from build123d import *

# Parameters (mm, degrees)
BASE_PLATE_PROFILE_SKETCH_R               = 4.1
BASE_PLATE_PROFILE_SKETCH_R_2             = 2.1
BASE_PLATE_7_5MM_DEPTH                    = 7.5
CONNECTOR_RECESS_26_4MM_X_2MM_DEPTH       = 2
CONNECTOR_BORE_AND_SCREW_HOLES_REACH      = 47.058
CONNECTOR_BORE_AND_SCREW_HOLES_SKETCH_R   = 8.05
CONNECTOR_BORE_AND_SCREW_HOLES_SKETCH_R_2 = 2.1


with BuildPart() as part:
    # Base Plate Profile Sketch → Base Plate 7.5mm (new body)
    with BuildSketch(Plane(origin=(0, 0, 0), x_dir=(1, 0, 0), z_dir=(0, 1, 0))):
        with BuildLine():
            Line((-34.1, 20), (-34.1, 18.5))
            ThreePointArc((-34.1, 18.5), (-30, 14.4), (-25.9, 18.5))
            Line((-25.9, 18.5), (-25.9, 20))
            Line((-25.9, 20), (25.9, 20))
            Line((25.9, 20), (25.9, 18.5))
            ThreePointArc((25.9, 18.5), (30, 14.4), (34.1, 18.5))
            Line((34.1, 18.5), (34.1, 20))
            Line((34.1, 20), (36, 20))
            ThreePointArc((36, 20), (38.828427125, 18.828427125), (40, 16))
            Line((40, 16), (40, -16))
            ThreePointArc((40, -16), (38.828427125, -18.828427125), (36, -20))
            Line((36, -20), (34.1, -20))
            Line((34.1, -20), (34.1, -18.5))
            ThreePointArc((34.1, -18.5), (30, -14.4), (25.9, -18.5))
            Line((25.9, -18.5), (25.9, -20))
            Line((25.9, -20), (-25.9, -20))
            Line((-25.9, -20), (-25.9, -18.5))
            ThreePointArc((-25.9, -18.5), (-30, -14.4), (-34.1, -18.5))
            Line((-34.1, -18.5), (-34.1, -20))
            Line((-34.1, -20), (-36, -20))
            ThreePointArc((-36, -20), (-38.828427125, -18.828427125), (-40, -16))
            Line((-40, -16), (-40, 16))
            ThreePointArc((-40, 16), (-38.828427125, 18.828427125), (-36, 20))
            Line((-36, 20), (-34.1, 20))
        make_face()
        with Locations(Location((-30, 0, 0), (0, 0, 270))):
            Circle(BASE_PLATE_PROFILE_SKETCH_R, mode=Mode.SUBTRACT)
        with Locations(Location((30, 0, 0), (0, 0, 90))):
            Circle(BASE_PLATE_PROFILE_SKETCH_R, mode=Mode.SUBTRACT)
        with Locations(Location((-20, 0, 0), (0, 0, 270))):
            Circle(BASE_PLATE_PROFILE_SKETCH_R_2, mode=Mode.SUBTRACT)
        with Locations(Location((20, 0, 0), (0, 0, 90))):
            Circle(BASE_PLATE_PROFILE_SKETCH_R_2, mode=Mode.SUBTRACT)
    extrude(amount=BASE_PLATE_7_5MM_DEPTH)

    # Connector Recess Sketch → Connector Recess 26.4mm x 2mm (cut)
    with BuildSketch(Plane(origin=(0, 7.5, 0), x_dir=(1, 0, 0), z_dir=(0, 1, 0))):
        with BuildLine():
            Line((-9.2, -13.2), (9.2, -13.2))
            ThreePointArc((9.2, -13.2), (12.028427125, -12.028427125), (13.2, -9.2))
            Line((13.2, -9.2), (13.2, 9.2))
            ThreePointArc((13.2, 9.2), (12.028427125, 12.028427125), (9.2, 13.2))
            Line((9.2, 13.2), (-9.2, 13.2))
            ThreePointArc((-9.2, 13.2), (-12.028427125, 12.028427125), (-13.2, 9.2))
            Line((-13.2, 9.2), (-13.2, -9.2))
            ThreePointArc((-13.2, -9.2), (-12.028427125, -12.028427125), (-9.2, -13.2))
        make_face()
    extrude(amount=-CONNECTOR_RECESS_26_4MM_X_2MM_DEPTH, mode=Mode.SUBTRACT)

    # Connector Bore and Screw Holes Sketch → Connector Bore and Screw Holes (cut, up to next)
    with BuildSketch(Plane(origin=(0, 5.5, 0), x_dir=(1, 0, 0), z_dir=(0, 1, 0)), mode=Mode.PRIVATE) as connector_bore_and_screw_holes_sk1:
        with Locations(Location((0, 0, 0), (0, 0, 270))):
            Circle(CONNECTOR_BORE_AND_SCREW_HOLES_SKETCH_R)
    connector_bore_and_screw_holes_tool1 = extrude(connector_bore_and_screw_holes_sk1.sketch, amount=-CONNECTOR_BORE_AND_SCREW_HOLES_REACH, mode=Mode.PRIVATE) & part.part
    # Connector Bore and Screw Holes Sketch → Connector Bore and Screw Holes (cut, up to next)
    with BuildSketch(Plane(origin=(0, 5.5, 0), x_dir=(1, 0, 0), z_dir=(0, 1, 0)), mode=Mode.PRIVATE) as connector_bore_and_screw_holes_sk2:
        with Locations(Location((-9.2, 9.2, 0), (0, 0, 270))):
            Circle(CONNECTOR_BORE_AND_SCREW_HOLES_SKETCH_R_2)
    connector_bore_and_screw_holes_tool2 = extrude(connector_bore_and_screw_holes_sk2.sketch, amount=-CONNECTOR_BORE_AND_SCREW_HOLES_REACH, mode=Mode.PRIVATE) & part.part
    # Connector Bore and Screw Holes Sketch → Connector Bore and Screw Holes (cut, up to next)
    with BuildSketch(Plane(origin=(0, 5.5, 0), x_dir=(1, 0, 0), z_dir=(0, 1, 0)), mode=Mode.PRIVATE) as connector_bore_and_screw_holes_sk3:
        with Locations(Location((-9.2, -9.2, 0), (0, 0, 270))):
            Circle(CONNECTOR_BORE_AND_SCREW_HOLES_SKETCH_R_2)
    connector_bore_and_screw_holes_tool3 = extrude(connector_bore_and_screw_holes_sk3.sketch, amount=-CONNECTOR_BORE_AND_SCREW_HOLES_REACH, mode=Mode.PRIVATE) & part.part
    # Connector Bore and Screw Holes Sketch → Connector Bore and Screw Holes (cut, up to next)
    with BuildSketch(Plane(origin=(0, 5.5, 0), x_dir=(1, 0, 0), z_dir=(0, 1, 0)), mode=Mode.PRIVATE) as connector_bore_and_screw_holes_sk4:
        with Locations(Location((9.2, -9.2, 0), (0, 0, 270))):
            Circle(CONNECTOR_BORE_AND_SCREW_HOLES_SKETCH_R_2)
    connector_bore_and_screw_holes_tool4 = extrude(connector_bore_and_screw_holes_sk4.sketch, amount=-CONNECTOR_BORE_AND_SCREW_HOLES_REACH, mode=Mode.PRIVATE) & part.part
    # Connector Bore and Screw Holes Sketch → Connector Bore and Screw Holes (cut, up to next)
    with BuildSketch(Plane(origin=(0, 5.5, 0), x_dir=(1, 0, 0), z_dir=(0, 1, 0)), mode=Mode.PRIVATE) as connector_bore_and_screw_holes_sk5:
        with Locations(Location((9.2, 9.2, 0), (0, 0, 270))):
            Circle(CONNECTOR_BORE_AND_SCREW_HOLES_SKETCH_R_2)
    connector_bore_and_screw_holes_tool5 = extrude(connector_bore_and_screw_holes_sk5.sketch, amount=-CONNECTOR_BORE_AND_SCREW_HOLES_REACH, mode=Mode.PRIVATE) & part.part
    add(connector_bore_and_screw_holes_tool1.solids().sort_by_distance((0, 5.5, 0))[0], mode=Mode.SUBTRACT)
    add(connector_bore_and_screw_holes_tool2.solids().sort_by_distance((-9.2, 5.5, -9.2))[0], mode=Mode.SUBTRACT)
    add(connector_bore_and_screw_holes_tool3.solids().sort_by_distance((-9.2, 5.5, 9.2))[0], mode=Mode.SUBTRACT)
    add(connector_bore_and_screw_holes_tool4.solids().sort_by_distance((9.2, 5.5, 9.2))[0], mode=Mode.SUBTRACT)
    add(connector_bore_and_screw_holes_tool5.solids().sort_by_distance((9.2, 5.5, -9.2))[0], mode=Mode.SUBTRACT)


solid = part.part
CAD build for the part. Positions are in the model's coordinates, mm. A direction names the side the tool comes from. Give positions to 0.01 mm unless a question says otherwise; leave off trailing zeros. Write each loop counter-clockwise with the first axis right and the second up, starting at its lowest first coordinate (ties: lowest second). Pieces come first, ordered by that corner, then holes. Notation, with made-up numbers: (19.25, 2) - (30.25, 2) arc R18 ccw to (30.25, 23) - close; hole circle Ø5 at (14, -13.75). An arc over 180 degrees is marked (long way). Put each result on its own line as item: value.
(1) Saw through at D-D (z = 3). List the corners of the cut face in (x, y).
Working result:
outline: (-40, 0) - (-32.79, 0) - (-32.79, 7.5) - (-40, 7.5) - close; (-27.21, 0) - (-7.47, 0) - (-7.47, 5.5) - (-13.2, 5.5) - (-13.2, 7.5) - (-27.21, 7.5) - close; (7.47, 0) - (27.21, 0) - (27.21, 7.5) - (13.2, 7.5) - (13.2, 5.5) - (7.47, 5.5) - close; (32.79, 0) - (40, 0) - (40, 7.5) - (32.79, 7.5) - close
(2) Tool access for faces 5 (the flat face through (34.1, 4, 19)), 6 (the flat face through (0, 7, -13.2)), 7 (the flat face through (-25.9, 4, -19)): list every direction of +Z, -Z, +X, -X, +Y, -Y with a clear straight run to the whole face (end or side of a thin tool).
Working result:
face 5: +Z, +Y, -Y
face 6: +Y
face 7: -Z, +Y, -Y
(3) Saw through at C-C (x = 30). List the corners of the cut face in (y, z), then the cut area to 4 significant figures.
Working result:
outline: (0, -14.4) - (7.5, -14.4) - (7.5, -4.1) - (0, -4.1) - close; (0, 4.1) - (7.5, 4.1) - (7.5, 14.4) - (0, 14.4) - close
area: 154.5 mm^2
(4) Saw through at A-A (x = -20). List the corners of the cut face in (y, z), then the cut area to 4 significant figures.
Working result:
outline: (0, -20) - (7.5, -20) - (7.5, -2.1) - (0, -2.1) - close; (0, 2.1) - (7.5, 2.1) - (7.5, 20) - (0, 20) - close
area: 268.5 mm^2
(5) Saw through at B-B (y = 2.25). Count the separate pieces of the cut face and the enclosed holes in it, then the cut area to 3 significant figures.
Working result:
separate pieces: 1
enclosed holes: 9
area: 2,640 mm^2
(6) Pull direction Z, two halves, no side cores. Call faces 1 (the flat face through (35, 4, -20)), 2 (the cylindrical face through (-3.083, 2.788, 7.436)), 3 (the cylindrical face through (-29.9, 3.7, 14.4)), 4 (the flat face through (25.9, 4, 19)): released by +Z, released by -Z, zero draft, split by the parting line, or undercut.
Working result:
face 1: released by -Z
face 2: undercut
face 3: released by +Z
face 4: zero draft
(7) Drop flat-ended pins along their axis: pin 1 Ø1.6 at (y, z) = (3.5, -19.5) entering from +X; pin 2 Ø1.2 at (y, z) = (5, 19) entering from +X; pin 3 Ø4 at (x, z) = (9.2, 9.2) entering from +Y; pin 4 Ø21 at (x, z) = (0, 0) entering from +Y. Give the stop position or say it passes through.
Working result:
pin 1: x = 38.95
pin 2: x = 39.2
pin 3: through
pin 4: y = 5.5
(8) Wall check: L1, parallel to X at y = 1.75, z = 9; L2, parallel to X at y = 3.75, z = 0; L3, parallel to Z at x = -0.5, y = 4.75. Give the ranges that are in metal, low to high.
Working result:
L1: -40 to -11.29, -7.11 to 7.11, 11.29 to 40
L2: -40 to -34.1, -25.9 to -22.1, -17.9 to -8.05, 8.05 to 17.9, 22.1 to 25.9, 34.1 to 40
L3: -20 to -8.03, 8.03 to 20
